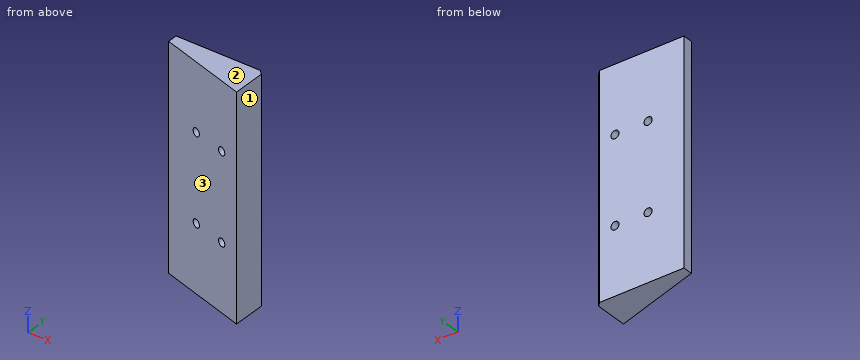
from build123d import *

# Parameters (mm, degrees)
BOSS_EXTRUDE1_DEPTH = 280
M12_TAPPED_HOLE1_D  = 10.2


with BuildPart() as part:
    # Sketch1 → Boss-Extrude1 (new body)
    with BuildSketch(Plane.XY):
        Polygon((0, 0), (0, 12.5), (107, 12.5), (112, 7.5), (112, -34.2), align=None)
    extrude(amount=BOSS_EXTRUDE1_DEPTH)

    # M12 Tapped Hole1 (through all)
    with Locations(Plane(origin=(0, 12.5, 0), x_dir=(-1, 0, 0), z_dir=(0, 1, 0))):
        with Locations((-45.5, 195), (-45.5, 85), (-87.5, 85), (-87.5, 195)):
            Hole(M12_TAPPED_HOLE1_D / 2)


solid = part.part
For this review, take the finished solid that the model builds, in its own axes (mm). Face numbers are marked on the shaded views. Give positions to 0.01 mm unless a question says otherwise; leave off trailing zeros. Order: outer loops, then holes, each group sorted by start corner. A loop starts at its lowest first (then second) coordinate and runs counter-clockwise, first axis right, second up. Notation, with made-up numbers: M 16.25,35 L 40.25,35 A28 cw 40.25,64 Z; hole C 65.25,85.5 d7. An arc over 180 degrees is marked long. Answer in a Markdown table with one row per item. Add a question column.
(1) Wall thickness on probe 1 along Z at (x, y) = (87, -5); probe 2 along X at (y, z) = (2, 85); probe 3 along Z at (x, y) = (84, 9): over which ranges is each line inside the solid? List them lowest first. Write a range as [from, to].
(2) Consider section D-D on x = 45.5. State the section outline as (y, z) points.
(3) Consider section B-B on z = 85. State the section outline as (x, y) points.
(4) Mouldability with a two-part tool opening along X and no side actions: class the marked faces 1, 2 and 3 as +X half, -X half, draft (parallel to the pull), parting line (faces both ways), or undercut.
(5) Consider section C-C on y = -19. State the section outline as (x, z) points.
(6) Consider section A-A on x = 87.5. State the section outline as (y, z) points, and give its area (3 significant figures).
(7) For pin 1 (16.5 mm diameter, centred on x = 45.5, z = 85, fed in from -Y); pin 2 (10 mm diameter, centred on x = 42, z = 229, fed in from -Y); pin 3 (5 mm diameter, centred on x = 20.5, z = 229.5, fed in from -Y); pin 4 (8 mm diameter, centred on x = 87.5, z = 85, fed in from -Y), all flat-tipped, find the tip position at first contact; note any pin that passes through.
Evaluation:
| question | item | result |
|---|---|---|
| 1 | probe 1 | z = [0, 79.92], [90.08, 189.92], [200.08, 280] |
| 1 | probe 2 | x = [0, 40.4], [50.6, 82.4], [92.6, 112] |
| 1 | probe 3 | z = [0, 81.29], [88.71, 191.29], [198.71, 280] |
| 2 | outline | M -13.89,0 L 12.5,0 L 12.5,79.9 L -13.89,79.9 Z; M -13.89,90.1 L 12.5,90.1 L 12.5,189.9 L -13.89,189.9 Z; M -13.89,200.1 L 12.5,200.1 L 12.5,280 L -13.89,280 Z |
| 3 | outline | M 0,0 L 40.4,-12.34 L 40.4,12.5 L 0,12.5 Z; M 50.6,-15.45 L 82.4,-25.16 L 82.4,12.5 L 50.6,12.5 Z; M 92.6,-28.28 L 112,-34.2 L 112,7.5 L 107,12.5 L 92.6,12.5 Z |
| 4 | face 1 | +X half |
| 4 | face 2 | draft |
| 4 | face 3 | -X half |
| 5 | outline | M 62.22,0 L 112,0 L 112,280 L 62.22,280 Z; hole C 87.5,85 d10.2; hole C 87.5,195 d10.2 |
| 6 | outline | M -26.72,0 L 12.5,0 L 12.5,79.9 L -26.72,79.9 Z; M -26.72,90.1 L 12.5,90.1 L 12.5,189.9 L -26.72,189.9 Z; M -26.72,200.1 L 12.5,200.1 L 12.5,280 L -26.72,280 Z |
| 6 | area | 10,200 mm^2 |
| 7 | pin 1 | stops at y = -16.41 |
| 7 | pin 2 | stops at y = -14.35 |
| 7 | pin 3 | stops at y = -7.02 |
| 7 | pin 4 | passes through |
